The listing builds one solid part. Answer for the finished solid, in the listing's coordinates (mm). Coordinates: 2 decimals unless noted, no trailing zeros. Order: outer loops, then holes, each group sorted by start corner. A loop starts at its lowest first (then second) coordinate and runs counter-clockwise, first axis right, second up. Notation, with made-up numbers: (27, -33) - (81, -33) arc R15 cw to (81, -14) - close; hole circle Ø3 at (-16.5, 66). An arc over 180 degrees is marked (long way). Use a Markdown table: item, result. Add a question column.
Item 1: The part is cut by section B-B, the plane x = 0. Give the vertices of the cut face in (y, z).
Item 2: The part is cut by section C-C, the plane z = 4.6. State how many separate pieces and enclosed holes the cut face has, then the cut area to 3 significant figures.
Item 3: Find the intervals of material crossed by line 1 along Y through (x, z) = (0, 4.15); line 2 along Y through (x, z) = (32.5, 1.4); line 3 along X through (y, z) = (7, 1.9), in increasing order.
Item 4: The part is cut by section A-A, the plane x = -30. Give the vertices of the cut face in (y, z).
Item 5: The part is cut by section D-D, the plane y = -9. Give the vertices of the cut face in (x, z), then the cut area to 3 significant figures.
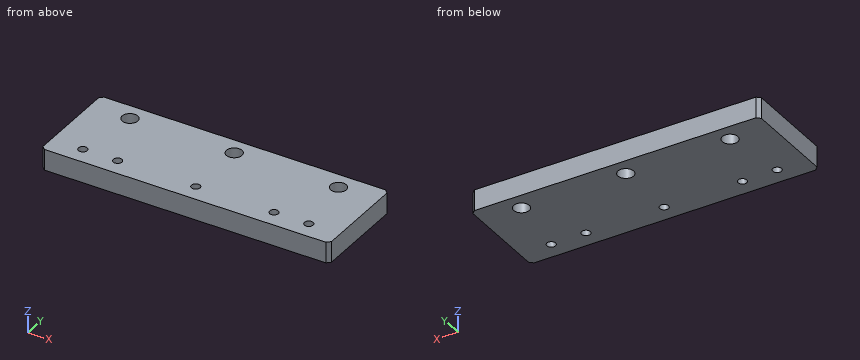
from build123d import *

# Parameters (mm, degrees)
SKETCH_1_W         = 83
SKETCH_1_H         = 28
EXTRUDE_1_DEPTH    = 6
HOLE_WIZARD_M4_1_D = 4.5
HOLE_WIZARD_M3_1_D = 2.5
CHAMFER_1_SIZE     = 1


with BuildPart() as part:
    # 草图1 → 凸台-拉伸1 (new body)
    with BuildSketch(Plane.XY):
        Rectangle(SKETCH_1_W, SKETCH_1_H)
    extrude(amount=EXTRUDE_1_DEPTH)

    # M4 间隙孔1 (through all)
    with Locations(Plane.XY.offset(6)):
        with Locations((-30, 9), (0, 9), (30, 9)):
            Hole(HOLE_WIZARD_M4_1_D / 2)

    # M3 螺纹孔1 (through all)
    with Locations(Plane.XY.offset(6)):
        with Locations((-32.5, -9), (0, -9), (32.5, -9), (22.5, -9), (-22.5, -9)):
            Hole(HOLE_WIZARD_M3_1_D / 2)

    # 倒角1
    chamfer_1_edges = [part.edges().sort_by_distance(p)[0] for p in [
        (41.5, -14, 3),
        (-41.5, -14, 3),
        (-41.5, 14, 3),
        (41.5, 14, 3),
    ]]
    chamfer(chamfer_1_edges, length=CHAMFER_1_SIZE)


solid = part.part
Solution:
| question | item | result |
|---|---|---|
| 1 | outline | (-14, 0) - (-10.25, 0) - (-10.25, 6) - (-14, 6) - close; (-7.75, 0) - (6.75, 0) - (6.75, 6) - (-7.75, 6) - close; (11.25, 0) - (14, 0) - (14, 6) - (11.25, 6) - close |
| 2 | separate pieces | 1 |
| 2 | enclosed holes | 8 |
| 2 | area | 2,250 mm2 |
| 3 | line 1 | y = -14 to -10.25, -7.75 to 6.75, 11.25 to 14 |
| 3 | line 2 | y = -14 to -10.25, -7.75 to 14 |
| 3 | line 3 | x = -41.5 to -31.03, -28.97 to -1.03, 1.03 to 28.97, 31.03 to 41.5 |
| 4 | outline | (-14, 0) - (6.75, 0) - (6.75, 6) - (-14, 6) - close; (11.25, 0) - (14, 0) - (14, 6) - (11.25, 6) - close |
| 5 | outline | (-41.5, 0) - (-33.75, 0) - (-33.75, 6) - (-41.5, 6) - close; (-31.25, 0) - (-23.75, 0) - (-23.75, 6) - (-31.25, 6) - close; (-21.25, 0) - (-1.25, 0) - (-1.25, 6) - (-21.25, 6) - close; (1.25, 0) - (21.25, 0) - (21.25, 6) - (1.25, 6) - close; (23.75, 0) - (31.25, 0) - (31.25, 6) - (23.75, 6) - close; (33.75, 0) - (41.5, 0) - (41.5, 6) - (33.75, 6) - close |
| 5 | area | 423 mm2 |
